The model under review builds one solid part; all positions refer to its coordinate system, in mm. Face numbers are marked on the shaded views. A direction names the side the tool comes from. Round coordinates to 2 decimals unless told otherwise and drop trailing zeros. Order: outer loops, then holes, each group sorted by start corner. A loop starts at its lowest first (then second) coordinate and runs counter-clockwise, first axis right, second up.
from build123d import *

# Parameters (mm, degrees)
BASE_PROFILE_SKETCH_R        = 10
BASE_PROFILE_SKETCH_R_2      = 6.25
BASE_PLATE_3MM_DEPTH         = 3
MOUNTING_WEB_6MM_DEPTH       = 6
BASE_START                   = -13
SKETCH1_4_R                  = 10
SKETCH1_4_R_2                = 6.25
BASE_BLOCK_13MM_DEPTH        = 13
SIDE_WALL_SKETCH_W           = 50
SIDE_WALL_SKETCH_H           = 55
SIDE_WALL_6MM_DEPTH          = 6
GUSSET_PROFILE_SKETCH_W      = 50
GUSSET_PROFILE_SKETCH_H      = 34
GUSSET_PROFILE_SKETCH_R      = 4
GUSSET_A_6MM_DEPTH           = 6
GUSSET_START                 = -49
SKETCH3_2_W                  = 50
SKETCH3_2_H                  = 34
SKETCH3_2_R                  = 4
GUSSET_B_6MM_DEPTH           = 6
CLEVIS_EYE_SKETCH_R          = 10
CLEVIS_EYE_SKETCH_R_2        = 5
CLEVIS_EYE_ARM_6MM_DEPTH     = 6
SKETCH4_3_R                  = 10
SKETCH4_3_R_2                = 5
CLEVIS_EYE_BOSS_A_10MM_DEPTH = 10
CLEVIS_START                 = 10
SKETCH4_4_R                  = 10
SKETCH4_4_R_2                = 5
CLEVIS_EYE_BOSS_B_10MM_DEPTH = 10
CLEVIS_PIVOT_BORE_SKETCH_R   = 6.25
CLEVIS_PIVOT_BORE_CUT_DEPTH  = 3
LOWER_PIVOT_BOSS_SKETCH_R    = 6.25
LOWER_PIVOT_BOSS_SKETCH_R_2  = 5
LOWER_PIVOT_BOSS_16MM_DEPTH  = 16
LOWER_START                  = -3
LOWER_PIVOT_BORE_SKETCH_R    = 6.25
LOWER_PIVOT_BORE_CUT_DEPTH   = 3
SUPPORT_RIB_3MM_DEPTH        = 1.5
SPOT_FACE_PAD_SKETCH_R       = 10
SPOT_FACE_PAD_0_5MM_DEPTH    = 0.5
PAD_START                    = -1
PAD_RECESS_SKETCH_R          = 6.25
PAD_RECESS_1MM_DEPTH         = 1
CLEVIS_EDGE_FILLET_R1_R      = 1
RIB_EDGE_FILLET_R3_R         = 3


with BuildPart() as part:
    # Base Profile Sketch → Base Plate 3mm (new body)
    with BuildSketch(Plane(origin=(0, 0, 0), x_dir=(1, 0, 0), z_dir=(0, 1, 0))):
        with Locations(Location((0, 0, 0), (0, 0, 270))):
            Circle(BASE_PROFILE_SKETCH_R)
        with Locations(Location((0, 0, 0), (0, 0, 270))):
            Circle(BASE_PROFILE_SKETCH_R_2, mode=Mode.SUBTRACT)
    extrude(amount=BASE_PLATE_3MM_DEPTH)



with BuildPart() as body_2:
    # Sketch1_3 → Mounting Web 6mm (new body)
    with BuildSketch(Plane(origin=(0, 0, 0), x_dir=(1, 0, 0), z_dir=(0, 1, 0))):
        with BuildLine():
            Line((25, 50), (-25, 50))
            Line((-25, 50), (-9.6, -2.8))
            ThreePointArc((-9.6, -2.8), (-1.414213562, 9.899494937), (10, 0))
            ThreePointArc((10, 0), (9.899494937, -1.414213562), (9.6, -2.8))
            Line((9.6, -2.8), (25, 50))
        make_face()
    extrude(amount=-MOUNTING_WEB_6MM_DEPTH)


with BuildPart() as part_1:
    add(part.part)

    add(body_2.part)  # Base Block 13mm merges body 2
    # Sketch1_4 → Base Block 13mm (add)
    with BuildSketch(Plane(origin=(0, 0, 0), x_dir=(1, 0, 0), z_dir=(0, 1, 0)).offset(BASE_START)):
        with Locations(Location((0, 0, 0), (0, 0, 270))):
            Circle(SKETCH1_4_R)
        with Locations(Location((0, 0, 0), (0, 0, 270))):
            Circle(SKETCH1_4_R_2, mode=Mode.SUBTRACT)
    extrude(amount=BASE_BLOCK_13MM_DEPTH)

    # Side Wall Sketch → Side Wall 6mm (add)
    with BuildSketch(Plane(origin=(0, 0, -50), x_dir=(-1, 0, 0), z_dir=(0, 0, -1))):
        with Locations((0, -12.5)):
            Rectangle(SIDE_WALL_SKETCH_W, SIDE_WALL_SKETCH_H)
    extrude(amount=SIDE_WALL_6MM_DEPTH)

    # Gusset Profile Sketch → Gusset A 6mm (add)
    with BuildSketch(Plane(origin=(0, 15, 0), x_dir=(1, 0, 0), z_dir=(0, 1, 0))):
        with Locations((0, 67)):
            Rectangle(GUSSET_PROFILE_SKETCH_W, GUSSET_PROFILE_SKETCH_H)
        with Locations(Location((-17, 74, 0), (0, 0, 270))):
            Circle(GUSSET_PROFILE_SKETCH_R, mode=Mode.SUBTRACT)
        with Locations(Location((17, 74, 0), (0, 0, 270))):
            Circle(GUSSET_PROFILE_SKETCH_R, mode=Mode.SUBTRACT)
    extrude(amount=-GUSSET_A_6MM_DEPTH)

    # Sketch3_2 → Gusset B 6mm (add)
    with BuildSketch(Plane(origin=(0, 15, 0), x_dir=(1, 0, 0), z_dir=(0, 1, 0)).offset(GUSSET_START)):
        with Locations((0, 67)):
            Rectangle(SKETCH3_2_W, SKETCH3_2_H)
        with Locations(Location((-17, 74, 0), (0, 0, 270))):
            Circle(SKETCH3_2_R, mode=Mode.SUBTRACT)
        with Locations(Location((17, 74, 0), (0, 0, 270))):
            Circle(SKETCH3_2_R, mode=Mode.SUBTRACT)
    extrude(amount=-GUSSET_B_6MM_DEPTH)

    # Clevis Eye Sketch → Clevis Eye Arm 6mm (add)
    # profile 1 of 2: a face of its own
    with BuildSketch(Plane.XZ.offset(40)):
        with BuildLine():
            Line((-9.6, 2.8), (-25, -50))
            Line((-25, -50), (25, -50))
            Line((25, -50), (9.6, 2.8))
            ThreePointArc((9.6, 2.8), (9.899494937, 1.414213562), (10, 0))
            ThreePointArc((10, 0), (-1.414213562, -9.899494937), (-9.6, 2.8))
        make_face()
    # profile 2 of 2: a face of its own
    with BuildSketch(Plane.XZ.offset(40)):
        with Locations(Location((0, 0, 0), (0, 0, 90))):
            Circle(CLEVIS_EYE_SKETCH_R)
        with Locations(Location((0, 0, 0), (0, 0, 270))):
            Circle(CLEVIS_EYE_SKETCH_R_2, mode=Mode.SUBTRACT)
    extrude(amount=-CLEVIS_EYE_ARM_6MM_DEPTH)

    # Sketch4_3 → Clevis Eye Boss A 10mm (add)
    with BuildSketch(Plane.XZ.offset(40)):
        with Locations(Location((0, 0, 0), (0, 0, 90))):
            Circle(SKETCH4_3_R)
        with Locations(Location((0, 0, 0), (0, 0, 270))):
            Circle(SKETCH4_3_R_2, mode=Mode.SUBTRACT)
    extrude(amount=-CLEVIS_EYE_BOSS_A_10MM_DEPTH)

    # Sketch4_4 → Clevis Eye Boss B 10mm (add)
    with BuildSketch(Plane.XZ.offset(40).offset(CLEVIS_START)):
        with Locations(Location((0, 0, 0), (0, 0, 90))):
            Circle(SKETCH4_4_R)
        with Locations(Location((0, 0, 0), (0, 0, 270))):
            Circle(SKETCH4_4_R_2, mode=Mode.SUBTRACT)
    extrude(amount=-CLEVIS_EYE_BOSS_B_10MM_DEPTH)

    # Clevis Pivot Bore Sketch → Clevis Pivot Bore Cut (cut)
    with BuildSketch(Plane.XZ.offset(50)):
        with Locations(Location((0, 0, 0), (0, 0, 90))):
            Circle(CLEVIS_PIVOT_BORE_SKETCH_R)
    extrude(amount=-CLEVIS_PIVOT_BORE_CUT_DEPTH, mode=Mode.SUBTRACT)

    # Lower Pivot Boss Sketch → Lower Pivot Boss 16mm (add)
    with BuildSketch(Plane.XZ.offset(13)):
        with Locations(Location((0, 0, 0), (0, 0, 270))):
            Circle(LOWER_PIVOT_BOSS_SKETCH_R)
        with Locations(Location((0, 0, 0), (0, 0, 270))):
            Circle(LOWER_PIVOT_BOSS_SKETCH_R_2, mode=Mode.SUBTRACT)
    extrude(amount=-LOWER_PIVOT_BOSS_16MM_DEPTH)

    # Lower Pivot Bore Sketch → Lower Pivot Bore Cut (cut)
    with BuildSketch(Plane(origin=(0, 3, 0), x_dir=(1, 0, 0), z_dir=(0, 1, 0)).offset(LOWER_START)):
        with Locations(Location((0, 0, 0), (0, 0, 90))):
            Circle(LOWER_PIVOT_BORE_SKETCH_R)
    extrude(amount=LOWER_PIVOT_BORE_CUT_DEPTH, mode=Mode.SUBTRACT)

    # Support Rib Sketch → Support Rib 3mm (add, symmetric)
    with BuildSketch(Plane(origin=(0, 0, 0), x_dir=(0, 0, -1), z_dir=(1, 0, 0))):
        Polygon((50, 15), (8.511959117, 3), (8.511959117, 0), (50, 0), align=None)
        Polygon((9.118743045, -9.5), (21, -9.5), (21, -31), (9.118743045, -31), (9.118743045, -34), (50, -34), (50, -6), (9.118743045, -6), align=None)
    extrude(amount=SUPPORT_RIB_3MM_DEPTH, both=True)

    # Spot Face Pad Sketch → Spot Face Pad 0.5mm (add)
    with BuildSketch(Plane(origin=(0, 3, 0), x_dir=(1, 0, 0), z_dir=(0, 1, 0))):
        with Locations(Location((0, 0, 0), (0, 0, 270))):
            Circle(SPOT_FACE_PAD_SKETCH_R)
    extrude(amount=SPOT_FACE_PAD_0_5MM_DEPTH)

    # Pad Recess Sketch → Pad Recess 1mm (cut)
    with BuildSketch(Plane(origin=(0, 3.5, 0), x_dir=(1, 0, 0), z_dir=(0, 1, 0)).offset(PAD_START)):
        with Locations(Location((0, 0, 0), (0, 0, 90))):
            Circle(PAD_RECESS_SKETCH_R)
    extrude(amount=PAD_RECESS_1MM_DEPTH, mode=Mode.SUBTRACT)

    # Clevis Edge Fillet R1
    clevis_edge_fillet_r1_edges = [part_1.edges().sort_by_distance(p)[0] for p in [
        (13.25, 0, -50),
        (-13.25, 0, -50),
        (-13.25, -34, -50),
        (13.25, -34, -50),
    ]]
    fillet(clevis_edge_fillet_r1_edges, radius=CLEVIS_EDGE_FILLET_R1_R)

    # Rib Edge Fillet R3
    rib_edge_fillet_r3_edges = [part_1.edges().sort_by_distance(p)[0] for p in [
        (0, -9.5, -21),
        (0, -31, -21),
    ]]
    fillet(rib_edge_fillet_r3_edges, radius=RIB_EDGE_FILLET_R3_R)


solid = part_1.part
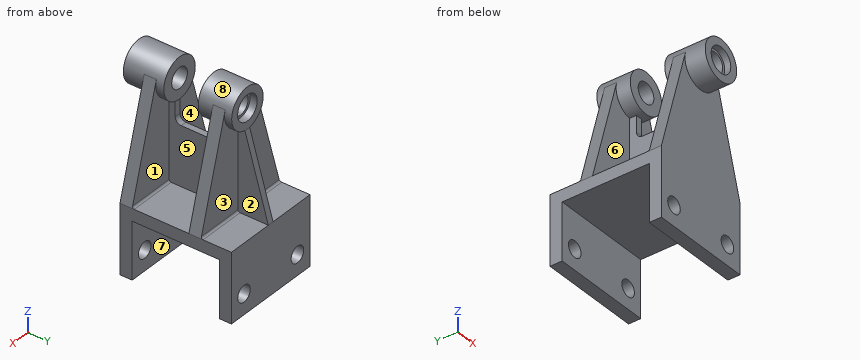
(1) We need section C-C (y = -3.5). Give the boundary of the cut face in (x, z), and give its area (3 significant figures).
(2) To check wall thickness, follow L1, parallel to X at y = -35.15, z = -74; L2, parallel to Y at x = 2, z = -74; L3, parallel to Y at x = -13, z = -32. State the ranges of each line that lie inside material, in increasing order.
(3) We need section B-B (x = -14). Give the boundary of the cut face in (y, z), and give its area (3 significant figures).
(4) The part is to be moulded in two halves that separate along Y. For the marked faces 1, 2, 3 and 4, say which applies: pulls with the +Y half, pulls with the -Y half, needs draft (parallel to the pull), parting line crosses it, or undercut.
(5) We need section D-D (y = -19.5). Give the boundary of the cut face in (x, z), and give its area (3 significant figures).
(6) Tool access review of the marked faces 5, 6, 7 and 8: name each direction out of +Z, -Z, +X, -X, +Y, -Y from which nothing blocks a thin tool from reaching the whole face with its end or side.
(7) We need section A-A (z = -63.5). Give the boundary of the cut face in (x, y), and give its area (3 significant figures).
(8) Clearance check with flat-ended pins moving along their axes: P1, Ø3, axis at x = 13, y = -28.5, coming from the -Z side; P2, Ø18.5, axis at x = -16, z = -19, coming from the +Y side; P3, Ø1, axis at y = 4.5, z = -43, coming from the -X side. State where each tip first meets the part, or that it passes through.
Verdict:
1. outline: (-25, -56) - (25, -56) - (25, -50) - (9.6, 2.8) arc R10 ccw to (-9.6, 2.8) - (-25, -50) - close; hole circle Ø10 at (0, 0)
1. area: 2,150 mm2
2. L1: x = -25 to -21, -13 to 13, 21 to 25
2. L2: y = -40 to -34, 9 to 15
2. L3: y = -40 to -34, -6 to 0
3. outline: (-40, -84) - (-34, -84) - (-34, -76.65) - (-40, -76.65) - close; (-40, -71.35) - (-34, -71.35) - (-34, -56) - (9, -56) - (9, -71.35) - (15, -71.35) - (15, -50) - (1, -50) arc R1 cw to (0, -49) - (0, -12.29) - (-6, -12.29) - (-6, -50) - (-33, -50) arc R1 cw to (-34, -49) - (-34, -12.29) - (-40, -12.29) - close; (9, -84) - (15, -84) - (15, -76.65) - (9, -76.65) - close
3. area: 1,060 mm2
4. face 1: undercut
4. face 2: needs draft
4. face 3: pulls with the +Y half
4. face 4: undercut
5. outline: (-25, -56) - (25, -56) - (25, -50) - (1.5, -50) - (1.5, -21) - (-1.5, -21) - (-1.5, -50) - (-25, -50) - close
5. area: 387 mm2
6. face 5: +X
6. face 6: -X
6. face 7: -Z, +X, -X
6. face 8: none
7. outline: (-25, -40) - (25, -40) - (25, -34) - (-25, -34) - close; (-25, 9) - (25, 9) - (25, 15) - (-25, 15) - close
7. area: 600 mm2
8. P1: stops at z = -56
8. P2: stops at y = 0
8. P3: stops at x = -1.5
